Can you work these out from the model? Positions are in its coordinate system, mm. A direction names the side the tool comes from. Round coordinates to 2 decimals unless told otherwise and drop trailing zeros. Order: outer loops, then holes, each group sorted by start corner. A loop starts at its lowest first (then second) coordinate and runs counter-clockwise, first axis right, second up.
Q1. We'd pull the mould along Y, two halves only. Please class faces 3 (the face through (1.97, -5.37, -1.19)), 4 (the face through (0.026, -3, 2)): pulls with the +Y half, pulls with the -Y half, needs draft (parallel to the pull), parting line crosses it, or undercut.
Q2. For faces 1 (the face through (2, -2, 0)), 2 (the face through (3.974, -3, -2)), which set-ups out of +Z, -Z, +X, -X, +Y, -Y let a thin tool reach every point of the face, with its end or its side?
Q3. If we section it at C-C (x = 0.95): Please give me the cut outline in (y, z), plus the area to 3 significant figures.
Q4. Will these pins go through, and if not, where does the flat tip stop? P1, Ø2.5, axis at y = 0, z = 0, coming from the +X side; P2, Ø1.5, axis at x = 1.5, y = -4, coming from the +Z side; P3, Ø1.5, axis at x = 3.5, z = 3.5, coming from the +Y side.
Q5. If I drill on line 1 (Y direction, x = 1.9, z = 0); line 2 (X direction, y = -3.5, z = -1.25); line 3 (Z direction, x = 1.7, y = 0.5), over which ranges is the centre line in solid material (lowest first)?
from build123d import *


with BuildPart() as part:
    # 草图1 → 旋转1 (revolve)
    with BuildSketch(Plane.XY, mode=Mode.PRIVATE) as revolve_1_sk:
        with BuildLine():
            Line((0, 5.35), (0, 4.555))
            Line((0, 4.555), (0.026, 4.555))
            Line((0.026, 4.555), (0.026, 3.2))
            Line((0.026, 3.2), (0, 3.2))
            Line((0, 3.2), (0, 2.15))
            ThreePointArc((0, 2.15), (0.043933983, 2.043933983), (0.15, 2))
            Line((0.15, 2), (3.85, 2))
            ThreePointArc((3.85, 2), (3.956066017, 2.043933983), (4, 2.15))
            Line((4, 2.15), (4, 3.2))
            Line((4, 3.2), (3.974, 3.2))
            Line((3.974, 3.2), (3.974, 4.555))
            Line((3.974, 4.555), (4, 4.555))
            Line((4, 4.555), (4, 5.35))
            ThreePointArc((4, 5.35), (3.956066017, 5.456066017), (3.85, 5.5))
            Line((3.85, 5.5), (0.15, 5.5))
            ThreePointArc((0.15, 5.5), (0.043933983, 5.456066017), (0, 5.35))
        make_face()
    revolve(revolve_1_sk.sketch.rotate(Axis((3.85, 0, 0), (-1, 0, 0)), 270), axis=Axis((3.85, 0, 0), (-1, 0, 0)))


solid = part.part
Solution:
1. face 3: parting line crosses it
1. face 4: undercut
2. face 1: +X, -X
2. face 2: +X
3. outline: circle Ø11 at (0, 0); hole circle Ø4 at (0, 0)
3. area: 82.5 mm2
4. P1: passes through
4. P2: stops at z = 4.44
4. P3: stops at y = 4.76
5. line 1: y = -5.5 to -2, 2 to 5.5
5. line 2: x = 0.03 to 3.97
5. line 3: z = -5.48 to -1.94, 1.94 to 5.48
